```python
from build123d import *

# Parameters (mm, degrees)
BASE_BODY_20MM_DEPTH       = 20
BASE_START                 = -14
BASE_SLOT_CUT_DEPTH        = 14
THIN_START                 = -68
THIN_WALL_BOSS_1_8MM_DEPTH = 68
JOURNAL_BLOCK_BOSS_DEPTH   = 69
JOURNAL_START              = -69
JOURNAL_BORE_CUT_DEPTH     = 69
JOURNAL_RELIEF_CUT_DEPTH   = 69
CROSS_ARM_BOSS_DEPTH       = 9
UPRIGHT_LUG_SKETCH_W       = 28
UPRIGHT_LUG_SKETCH_H       = 41
UPRIGHT_LUG_BOSS_DEPTH     = 35
LUG_START                  = -69
LUG_SLOT_CUT_DEPTH         = 69
SIDE_START                 = 18
SIDE_RIB_BOSS_DEPTH        = 18
BASE_EDGE_FILLET_R10_R     = 10


with BuildPart() as part:
    # Base Profile Sketch → Base Body 20mm (new body)
    with BuildSketch(Plane(origin=(0, 0, 0), x_dir=(0, 0, -1), z_dir=(1, 0, 0))):
        with BuildLine():
            Line((20.5, 0), (20.5, 7))
            Line((20.5, 7), (16, 7))
            Line((16, 7), (16, 14))
            ThreePointArc((16, 14), (0, 30), (-16, 14))
            Line((-16, 14), (-16, 7))
            Line((-16, 7), (-20.5, 7))
            Line((-20.5, 7), (-20.5, 0))
            Line((-20.5, 0), (-34.5, 0))
            Line((-34.5, 0), (-34.5, 21))
            ThreePointArc((-34.5, 21), (-30.399494937, 30.899494937), (-20.5, 35))
            Line((-20.5, 35), (34.5, 35))
            Line((34.5, 35), (34.5, 0))
            Line((34.5, 0), (20.5, 0))
        make_face()
    extrude(amount=BASE_BODY_20MM_DEPTH)

    # Base Slot Sketch → Base Slot Cut (cut)
    with BuildSketch(Plane(origin=(20, 0, 0), x_dir=(0, 0, -1), z_dir=(1, 0, 0)).offset(BASE_START)):
        with BuildLine():
            Line((-34.5, 14), (0, 35))
            Line((0, 35), (-20.5, 35))
            ThreePointArc((-20.5, 35), (-30.399494937, 30.899494937), (-34.5, 21))
            Line((-34.5, 21), (-34.5, 14))
        make_face()
    extrude(amount=BASE_SLOT_CUT_DEPTH, mode=Mode.SUBTRACT)

    # Thin Wall Profile Sketch → Thin Wall Boss 1.8mm (add)
    with BuildSketch(Plane(origin=(20, 0, 0), x_dir=(0, 0, -1), z_dir=(1, 0, 0)).offset(THIN_START)):
        with BuildLine():
            Line((-16, 14), (-16, 7))
            Line((-16, 7), (-20.5, 7))
            Line((-20.5, 7), (-20.5, 0))
            Line((-20.5, 0), (-22.3, 0))
            Line((-22.3, 0), (-22.3, 8.8))
            Line((-22.3, 8.8), (-17.8, 8.8))
            Line((-17.8, 8.8), (-17.8, 14))
            ThreePointArc((-17.8, 14), (0, 31.8), (17.8, 14))
            Line((17.8, 14), (17.8, 8.8))
            Line((17.8, 8.8), (22.3, 8.8))
            Line((22.3, 8.8), (22.3, 0))
            Line((22.3, 0), (20.5, 0))
            Line((20.5, 0), (20.5, 7))
            Line((20.5, 7), (16, 7))
            Line((16, 7), (16, 14))
            ThreePointArc((16, 14), (0, 30), (-16, 14))
        make_face()
    extrude(amount=THIN_WALL_BOSS_1_8MM_DEPTH)

    # Journal Block Sketch → Journal Block Boss (add)
    with BuildSketch(Plane.XY.offset(34.5)):
        with BuildLine():
            Line((-48, 0), (-28, 0))
            Line((-28, 0), (-28, 35))
            Line((-28, 35), (-34, 35))
            ThreePointArc((-34, 35), (-43.899494937, 30.899494937), (-48, 21))
            Line((-48, 21), (-48, 0))
        make_face()
    extrude(amount=-JOURNAL_BLOCK_BOSS_DEPTH)

    # Journal Bore Sketch → Journal Bore Cut (cut)
    with BuildSketch(Plane(origin=(20, 0, 0), x_dir=(0, 0, -1), z_dir=(1, 0, 0)).offset(JOURNAL_START)):
        with BuildLine():
            Line((-16, 14), (-16, 7))
            Line((-16, 7), (-20.5, 7))
            Line((-20.5, 7), (-20.5, 0))
            Line((-20.5, 0), (20.5, 0))
            Line((20.5, 0), (20.5, 7))
            Line((20.5, 7), (16, 7))
            Line((16, 7), (16, 14))
            ThreePointArc((16, 14), (0, 30), (-16, 14))
        make_face()
    extrude(amount=JOURNAL_BORE_CUT_DEPTH, mode=Mode.SUBTRACT)

    # Journal Relief Sketch → Journal Relief Cut (cut)
    with BuildSketch(Plane.XY.offset(34.5)):
        with BuildLine():
            Line((-48, 21), (-48, 35))
            Line((-48, 35), (-34, 35))
            ThreePointArc((-34, 35), (-43.899494937, 30.899494937), (-48, 21))
        make_face()
    extrude(amount=-JOURNAL_RELIEF_CUT_DEPTH, mode=Mode.SUBTRACT)

    # Cross Arm Sketch → Cross Arm Boss (add)
    with BuildSketch(Plane(origin=(0, 0, -34.5), x_dir=(-1, 0, 0), z_dir=(0, 0, -1))):
        with BuildLine():
            Line((48, 21), (48, 35))
            Line((48, 35), (48, 59))
            Line((48, 59), (48, 59.317541634))
            ThreePointArc((48, 59.317541634), (45.90569415, 65.441265991), (40.5, 69))
            Line((40.5, 69), (40.5, 49))
            ThreePointArc((40.5, 49), (34, 42.5), (27.5, 49))
            Line((27.5, 49), (27.5, 69))
            ThreePointArc((27.5, 69), (22.09430585, 65.441265991), (20, 59.317541634))
            Line((20, 59.317541634), (20, 21))
            Line((20, 21), (20, 0))
            Line((20, 0), (48, 0))
            Line((48, 0), (48, 21))
        make_face()
    extrude(amount=CROSS_ARM_BOSS_DEPTH)

    # Upright Lug Sketch → Upright Lug Boss (add)
    with BuildSketch(Plane(origin=(0, 35, 0), x_dir=(1, 0, 0), z_dir=(0, 1, 0))):
        with Locations((-14, 14)):
            Rectangle(UPRIGHT_LUG_SKETCH_W, UPRIGHT_LUG_SKETCH_H)
    extrude(amount=-UPRIGHT_LUG_BOSS_DEPTH)

    # Lug Slot Sketch → Lug Slot Cut (cut)
    with BuildSketch(Plane(origin=(20, 0, 0), x_dir=(0, 0, -1), z_dir=(1, 0, 0)).offset(LUG_START)):
        with BuildLine():
            Line((-16, 14), (-16, 7))
            Line((-16, 7), (-20.5, 7))
            Line((-20.5, 7), (-20.5, 0))
            Line((-20.5, 0), (20.5, 0))
            Line((20.5, 0), (20.5, 7))
            Line((20.5, 7), (16, 7))
            Line((16, 7), (16, 14))
            ThreePointArc((16, 14), (0, 30), (-16, 14))
        make_face()
    extrude(amount=LUG_SLOT_CUT_DEPTH, mode=Mode.SUBTRACT)

    # Side Rib Sketch → Side Rib Boss (add)
    with BuildSketch(Plane.XY.offset(-34.5).offset(SIDE_START)):
        with BuildLine():
            Line((-20, 35), (-20, 51))
            Line((-20, 51), (-27.5, 51))
            Line((-27.5, 51), (-27.5, 49))
            ThreePointArc((-27.5, 49), (-34, 42.5), (-40.5, 49))
            Line((-40.5, 49), (-40.5, 51))
            Line((-40.5, 51), (-48, 51))
            Line((-48, 51), (-48, 21))
            ThreePointArc((-48, 21), (-43.899494937, 30.899494937), (-34, 35))
            Line((-34, 35), (-20, 35))
        make_face()
    extrude(amount=-SIDE_RIB_BOSS_DEPTH)

    # Base Edge Fillet R10
    base_edge_fillet_r10_edges = [part.edges().sort_by_distance(p)[0] for p in [
        (20, 17.5, -34.5),
    ]]
    fillet(base_edge_fillet_r10_edges, radius=BASE_EDGE_FILLET_R10_R)


solid = part.part
```
Part model, mm, in its own coordinate system. A direction names the side the tool comes from. Round coordinates to 2 decimals unless told otherwise and drop trailing zeros. Order: outer loops, then holes, each group sorted by start corner. A loop starts at its lowest first (then second) coordinate and runs counter-clockwise, first axis right, second up. Notation, with made-up numbers: M -6.75,-18.75 L 52.25,-18.75 A22 cw 52.25,15.25 Z; hole C -14.5,78.5 d7. An arc over 180 degrees is marked long. Put each result on its own line as item: value. Start each with the question number.
1. Two-plate mould, pull along X, no slides. Class faces 1 (the face through (-28, 21, 24)), 2 (the face through (-33.9, 42.5, -29.8)), 3 (the face through (-38, 18, 34.5)), 4 (the face through (20, 26, 11)): +X half, -X half, draft (parallel to the pull), parting line (faces both ways), or undercut.
2. Slice it at A-A on y = 46.5. List the corners of the cut face in (x, z), then the cut area to 3 significant figures.
3. Slice it at B-B on x = -15.5. List the corners of the cut face in (y, z).
4. Slice it at C-C on z = 26. List the corners of the cut face in (x, y).
5. Tool access for faces 5 (the face through (6, 27, 21)), 6 (the face through (-14, 4, 22.3)), 7 (the face through (-44, 60, -34.5)): list every direction of +Z, -Z, +X, -X, +Y, -Y with a clear straight run to the whole face (end or side of a thin tool).
6. Drop flat-ended pins along their axis: pin 1 (4 mm diameter, centred on x = -23, z = -10, fed in from -Y); pin 2 (2 mm diameter, centred on y = 25.5, z = -7, fed in from -X); pin 3 (8 mm diameter, centred on x = -39, z = -1, fed in from +Y); pin 4 (1 mm diameter, centred on y = 36.5, z = -24.5, fed in from +X). Give the stop position or say it passes through.
7. Drill centre lines: probe 1 along X at (y, z) = (8, 23.5); probe 2 along Z at (x, y) = (-17, 5); probe 3 along X at (y, z) = (60, -35.5). Where is each one in solid material? Low to high. Write a range as [from, to].
8. Slice it at D-D on y = 11. List the corners of the cut face in (x, z).
Findings:
1. face 1: undercut
1. face 2: undercut
1. face 3: draft
1. face 4: +X half
2. outline: M -48,-43.5 L -40,-43.5 L -40,-16.5 L -48,-16.5 Z; M -28,-43.5 L -20,-43.5 L -20,-16.5 L -28,-16.5 Z
2. area: 432 mm2
3. outline: M 0,-34.5 L 35,-34.5 L 35,6.5 L 30.57,6.5 A17.8 ccw 14,17.8 L 8.8,17.8 L 8.8,22.3 L 0,22.3 L 0,20.5 L 7,20.5 L 7,16 L 14,16 A16 cw 14,-16 L 7,-16 L 7,-20.5 L 0,-20.5 Z
4. outline: M -48,0 L -28,0 L -28,35 L -34,35 A14 ccw -48,21 Z; M 0,0 L 20,0 L 20,19.17 L 6,19.17 L 6,33.87 L 0,33.87 Z
5. face 5: +Z, +X, +Y
5. face 6: +Z, +Y, -Y
5. face 7: +Z, +X, -X, +Y
6. pin 1: y = 24.58
6. pin 2: through
6. pin 3: y = 34.96
6. pin 4: x = -20
7. probe 1: [-48, -28], [0, 20]
7. probe 2: [-34.5, -20.5], [20.5, 22.3]
7. probe 3: [-47.98, -40.5], [-27.5, -20.02]
8. outline: M -48,-43.5 L -20,-43.5 L -20,-34.5 L 10,-34.5 A10 ccw 20,-24.5 L 20,-16 L -48,-16 Z; M -48,16 L 20,16 L 20,34.5 L 0,34.5 L 0,17.8 L -28,17.8 L -28,34.5 L -48,34.5 Z
